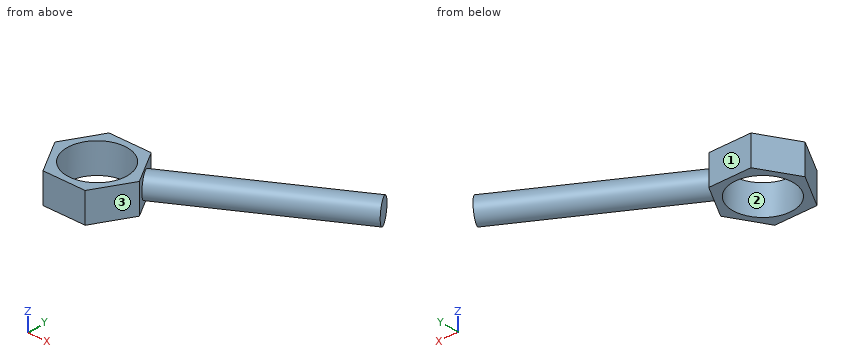
```python
from build123d import *

# Parameters (mm, degrees)
SKETCH1_R           = 5
BOSS_EXTRUDE1_DEPTH = 5
SKETCH2_R           = 2
BOSS_EXTRUDE2_DEPTH = 30


with BuildPart() as part:
    # Sketch1 → Boss-Extrude1 (new body)
    with BuildSketch(Plane.XY):
        Polygon((-3.5, 6.062177826), (-7, 0), (-3.5, -6.062177826), (3.5, -6.062177826), (7, 0), (3.5, 6.062177826), align=None)
        Circle(SKETCH1_R, mode=Mode.SUBTRACT)
    extrude(amount=BOSS_EXTRUDE1_DEPTH)

    # Sketch2 → Boss-Extrude2 (add)
    with BuildSketch(Plane(origin=(5.25, 3.031088913, 0), x_dir=(0, 0, -1), z_dir=(0.8660254037844387, 0.49999999999999983, 0))):
        with Locations(Location((-2.5, 0, 0), (0, 0, 90))):
            Circle(SKETCH2_R)
    extrude(amount=BOSS_EXTRUDE2_DEPTH)


solid = part.part
```
Design review of the part built by this model. Coordinates are the model's own, in mm. Face numbers are marked on the shaded views. Give positions to 0.01 mm unless a question says otherwise; leave off trailing zeros. Order: outer loops, then holes, each group sorted by start corner. A loop starts at its lowest first (then second) coordinate and runs counter-clockwise, first axis right, second up. Notation, with made-up numbers: (76, -20.5) -> (110, -20.5) arc R18 cw to (110, 0.5) -> close; hole circle Ø6 at (13.5, 4). An arc over 180 degrees is marked (long way). Write item = value, one per line. Start each with the question number.
(1) To check wall thickness, follow line 1 along Y through (x, z) = (0, 4); line 2 along X through (y, z) = (0.5, 1.75); line 3 along Y through (x, z) = (-2.5, 0.8). State the ranges of each line that lie inside material, in increasing order.
(2) We need section C-C on x = -4. Write out the cut boundary in (y, z), plus the area to 3 significant figures.
(3) Mouldability with a two-part tool opening along Y and no side actions: class the marked faces 1, 2 and 3 as +Y half, -Y half, draft (parallel to the pull), parting line (faces both ways), or undercut.
(4) For pin 1 (2 mm diameter, centred on x = 13.5, z = 1.5, fed in from +Y); pin 2 (10 mm diameter, centred on x = 11, y = 7, fed in from +Z); pin 3 (6 mm diameter, centred on x = 0, y = 0, fed in from +Z); pin 4 (6 mm diameter, centred on x = 22, y = 15, fed in from -Z), all flat-tipped, find the tip position at first contact; note any pin that passes through.
(5) We need section B-B on z = 2.9. Write out the cut boundary in (x, y), plus the area to 3 significant figures.
(6) We need section A-A on x = 0. Write out the cut boundary in (y, z).
Numbers:
q1.line_1 = -6.06 to -5, 5 to 6.06
q1.line_2 = -6.71 to -4.97, 4.97 to 6.71
q1.line_3 = -6.06 to -4.33, 4.33 to 6.06
q2.outline = (-5.2, 0) -> (-3, 0) -> (-3, 5) -> (-5.2, 5) -> close; (3, 0) -> (5.2, 0) -> (5.2, 5) -> (3, 5) -> close
q2.area = 22.0 mm^2
q3.face_1 = +Y half
q3.face_2 = undercut
q3.face_3 = -Y half
q4.pin_1 = 10.53
q4.pin_2 = 4.5
q4.pin_3 = through
q4.pin_4 = 0.5
q5.outline = (-7, 0) -> (-3.5, -6.06) -> (3.5, -6.06) -> (7, 0) -> (6.23, 1.33) -> (32.21, 16.33) -> (30.25, 19.73) -> (4.27, 4.73) -> (3.5, 6.06) -> (-3.5, 6.06) -> close; hole circle Ø10 at (0, 0)
q5.area = 166 mm^2
q6.outline = (-6.06, 0) -> (-5, 0) -> (-5, 5) -> (-6.06, 5) -> close; (5, 0) -> (6.06, 0) -> (6.06, 5) -> (5, 5) -> close
